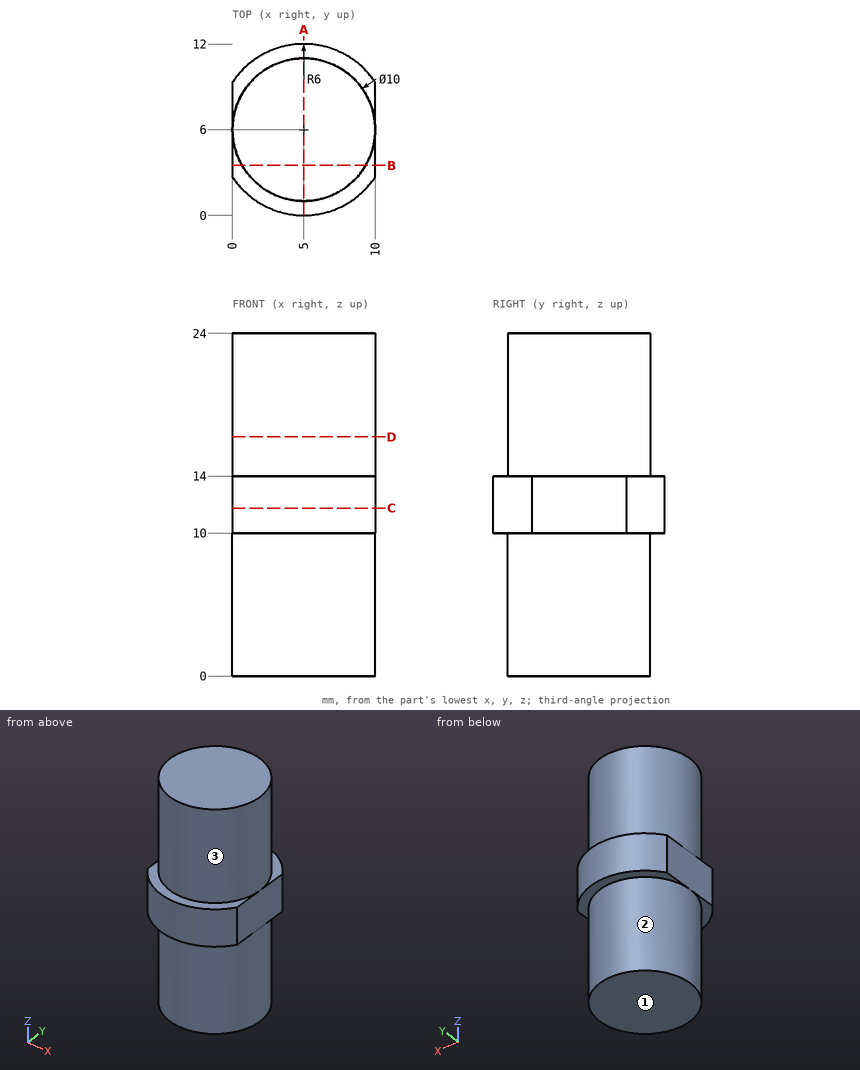
Design review of the part shown in the three views and the two pictorial views. Dimensions are in mm from the part's minimum x, y and z. A direction names the side the tool comes from. Coordinates: 2 decimals unless noted, no trailing zeros. Order: outer loops, then holes, each group sorted by start corner. A loop starts at its lowest first (then second) coordinate and runs counter-clockwise, first axis right, second up. Notation, with made-up numbers: (-12.75, 0) -> (21.25, 0) arc R23 ccw to (21.25, 26) -> close; hole circle Ø4 at (0, 69). An arc over 180 degrees is marked (long way). Use one line per item in the form item = value. Start each with the question number.
(1) Add section A-A on x = 5. State the section outline as (y, z) points, plus the area to 3 significant figures.
(2) Add section C-C on z = 11.75. State the section outline as (x, y) points, plus the area to 3 significant figures.
(3) Add section B-B on y = 3.5. State the section outline as (x, z) points, plus the area to 3 significant figures.
(4) Add section D-D on z = 16.75. State the section outline as (x, y) points, plus the area to 3 significant figures.
(5) Insertion check: pin 1 (3 mm diameter, centred on y = 8, z = 20.5, fed in from -X). The pin has a flat end and moves straight along its axis. Give the tip position at first contact, or say it passes through.
(6) For probe 1 along Y at (x, z) = (5, 17.5); probe 2 along Z at (x, y) = (5, 11.5); probe 3 along X at (y, z) = (8.5, 8.75), list the stretches that pass through material, from the lowest coordinate up.
(7) For the marked faces 1, 2 and 3, list the 3-axis set-ups (+Z, -Z, +X, -X, +Y, -Y) from which the entire face can be reached by the end or side of a thin tool; tool diameter is ignored.
Answer block:
q1.outline = (0, 10) -> (1, 10) -> (1, 0) -> (11, 0) -> (11, 10) -> (12, 10) -> (12, 14) -> (11, 14) -> (11, 24) -> (1, 24) -> (1, 14) -> (0, 14) -> close
q1.area = 248 mm²
q2.outline = (0, 2.68) arc R6 ccw to (10, 2.68) -> (10, 9.32) arc R6 ccw to (0, 9.32) -> close
q2.area = 104 mm²
q3.outline = (0, 10) -> (0.67, 10) -> (0.67, 0) -> (9.33, 0) -> (9.33, 10) -> (10, 10) -> (10, 14) -> (9.33, 14) -> (9.33, 24) -> (0.67, 24) -> (0.67, 14) -> (0, 14) -> close
q3.area = 213 mm²
q4.outline = circle Ø10 at (5, 6)
q4.area = 78.5 mm²
q5.pin_1 = 0.03
q6.probe_1 = 1 to 11
q6.probe_2 = 10 to 14
q6.probe_3 = 0.67 to 9.33
q7.face_1 = -Z, +X, -X, +Y, -Y
q7.face_2 = -Z
q7.face_3 = +Z
